Source: CAD feature listing. Evaluate the final solid. Frame: model axes, mm. Coordinates: 2 decimals unless noted, no trailing zeros. Loops run counter-clockwise (first coordinate to the right, second up) from the corner with the lowest first, then second, coordinate; pieces in that order, holes last. Notation, with made-up numbers: (69, 25) -> (110, 25) arc R12 ccw to (110, 29) -> close; hole circle Ø3 at (10.5, 29.25). An arc over 180 degrees is marked (long way). Answer as CSV lines item,"result".
from build123d import *

# Parameters (mm, degrees)
EXTRUDE_1_DEPTH     = 20.25
SKETCH_2_R          = 5
CUT_EXTRUDE_1_DEPTH = 52.5


with BuildPart() as part:
    # 草图1 → 凸台-拉伸1 (new, symmetric)
    with BuildSketch(Plane.XY):
        Polygon((0, 0), (550.66, 0), (545.33, -45.55), (275.33, -45.55), (5.33, -45.55), align=None)
    extrude(amount=EXTRUDE_1_DEPTH, both=True)

    # 草图2 → 切除-拉伸1 (cut)
    with BuildSketch(Plane(origin=(0, 0, 0), x_dir=(1, 0, 0), z_dir=(0, 1, 0))):
        with Locations(Location((535.33, 3.62, 0), (0, 0, 270))):
            Circle(SKETCH_2_R)
        with Locations(Location((275.33, 3.62, 0), (0, 0, 270))):
            Circle(SKETCH_2_R)
        with Locations(Location((15.33, 3.62, 0), (0, 0, 270))):
            Circle(SKETCH_2_R)
    extrude(amount=-CUT_EXTRUDE_1_DEPTH, mode=Mode.SUBTRACT)


solid = part.part
(1) Cut plane C-C (y = -15). Return the cut outline in (x, z), then the cut area to 3 significant figures.
Computed values:
outline,"(1.76, -20.25) -> (548.9, -20.25) -> (548.9, 20.25) -> (1.76, 20.25) -> close; hole circle Ø10 at (15.33, -3.62); hole circle Ø10 at (275.33, -3.62); hole circle Ø10 at (535.33, -3.62)"
area,"21,900 mm^2"
(2) Pin query (flat end, axial travel): pin 1 Ø4 at (y, z) = (-8, 2) entering from -X; pin 2 Ø10 at (y, z) = (-34.5, 2) entering from -X; pin 3 Ø1.5 at (y, z) = (-31, -7.5) entering from +X. Return the tip coordinate at first contact, or that it passes through.
Computed values:
pin 1,"x = 0.7"
pin 2,"x = 3.45"
pin 3,"x = 547.12"
(3) Material intervals for L1, parallel to X at y = -36, z = -3; L2, parallel to X at y = -9, z = -3.5; L3, parallel to Z at x = 275.33, y = -16, sorted ascending. Write a range as [from, to].
Computed values:
L1,"[4.21, 10.37], [20.29, 270.37], [280.29, 530.37], [540.29, 546.45]"
L2,"[1.05, 10.33], [20.33, 270.33], [280.33, 530.33], [540.33, 549.61]"
L3,"[-20.25, -8.62], [1.38, 20.25]"
(4) Cut plane D-D (y = -37.5). Return the cut outline in (x, z).
Computed values:
outline,"(4.39, -20.25) -> (546.27, -20.25) -> (546.27, 20.25) -> (4.39, 20.25) -> close; hole circle Ø10 at (15.33, -3.62); hole circle Ø10 at (275.33, -3.62); hole circle Ø10 at (535.33, -3.62)"
(5) Cut plane A-A (z = -3.62). Return the cut outline in (x, y), then the cut area to 3 significant figures.
Computed values:
outline,"(0, 0) -> (5.33, -45.55) -> (10.33, -45.55) -> (10.33, 0) -> close; (20.33, -45.55) -> (270.33, -45.55) -> (270.33, 0) -> (20.33, 0) -> close; (280.33, -45.55) -> (530.33, -45.55) -> (530.33, 0) -> (280.33, 0) -> close; (540.33, -45.55) -> (545.33, -45.55) -> (550.66, 0) -> (540.33, 0) -> close"
area,"23,500 mm^2"
(6) Draft query along X for faces 1 (the flat face through (548.03, -22.46, 0.28)), 2 (the flat face through (2.7, -23.09, 0.28)), 3 (the cylindrical face through (540.287, -22.456, -4.271)), 4 (the flat face through (271.6, -45.55, 0.3)). Return one class per face: released by +X, released by -X, zero draft, split by the parting line, or undercut.
Computed values:
face 1,"released by +X"
face 2,"released by -X"
face 3,"undercut"
face 4,"zero draft"
(7) Cut plane B-B (x = 535.33). Return the cut outline in (y, z).
Computed values:
outline,"(-45.55, -20.25) -> (0, -20.25) -> (0, -8.62) -> (-45.55, -8.62) -> close; (-45.55, 1.38) -> (0, 1.38) -> (0, 20.25) -> (-45.55, 20.25) -> close"
